from build123d import *

# Parameters (mm, degrees)
EXTRUDE_1_DEPTH     = 2
SKETCH_3_W          = 35
SKETCH_3_H          = 2
EXTRUDE_2_DEPTH     = 18
CUT_EXTRUDE_1_REACH = 87.112
SKETCH_4_R          = 2.5


with BuildPart() as part:
    # 草图1 → 旋转1 (revolve)
    with BuildSketch(Plane.XY):
        Polygon((0, 30), (0, 18.550632587), (0, 0), (18, 0), (18, 30), (15, 30), (15, 26), (3, 26), (3, 30), align=None)
    revolve(axis=Axis((18, 0, 0), (-1, 0, 0)))

    # 草图2 → 凸台-拉伸1 (add)
    with BuildSketch(Plane(origin=(18, 0, 0), x_dir=(0, 0, -1), z_dir=(1, 0, 0))):
        with BuildLine():
            Line((17.5, -40), (17.5, 0))
            ThreePointArc((17.5, 0), (0, 17.5), (-17.5, 0))
            Line((-17.5, 0), (-17.5, -40))
            Line((-17.5, -40), (17.5, -40))
        make_face()
    extrude_1 = extrude(amount=EXTRUDE_1_DEPTH)

    # 草图3 → 凸台-拉伸2 (add)
    with BuildSketch(Plane(origin=(20, 0, 0), x_dir=(0, 0, -1), z_dir=(1, 0, 0))):
        with Locations((0, -39)):
            Rectangle(SKETCH_3_W, SKETCH_3_H)
    extrude_2 = extrude(amount=EXTRUDE_2_DEPTH)

    # 镜向1: 凸台-拉伸1, 凸台-拉伸2 across plane
    add(extrude_1.mirror(Plane(origin=(9, 0, 0), x_dir=(0, 0, 1), z_dir=(1, 0, 0))))
    add(extrude_2.mirror(Plane(origin=(9, 0, 0), x_dir=(0, 0, 1), z_dir=(1, 0, 0))))

    # 草图4 → 切除-拉伸1 (cut, up to next)
    with BuildSketch(Plane.XZ.offset(40), mode=Mode.PRIVATE) as cut_extrude_1_sk1:
        with Locations((-12.5, 11)):
            Circle(SKETCH_4_R)
    cut_extrude_1_tool1 = extrude(cut_extrude_1_sk1.sketch, amount=-CUT_EXTRUDE_1_REACH, mode=Mode.PRIVATE) & part.part
    # 草图4 → 切除-拉伸1 (cut, up to next)
    with BuildSketch(Plane.XZ.offset(40), mode=Mode.PRIVATE) as cut_extrude_1_sk2:
        with Locations(Location((-12.5, -11, 0), (0, 0, 180))):
            Circle(SKETCH_4_R)
    cut_extrude_1_tool2 = extrude(cut_extrude_1_sk2.sketch, amount=-CUT_EXTRUDE_1_REACH, mode=Mode.PRIVATE) & part.part
    # 草图4 → 切除-拉伸1 (cut, up to next)
    with BuildSketch(Plane.XZ.offset(40), mode=Mode.PRIVATE) as cut_extrude_1_sk3:
        with Locations((30.5, -11)):
            Circle(SKETCH_4_R)
    cut_extrude_1_tool3 = extrude(cut_extrude_1_sk3.sketch, amount=-CUT_EXTRUDE_1_REACH, mode=Mode.PRIVATE) & part.part
    # 草图4 → 切除-拉伸1 (cut, up to next)
    with BuildSketch(Plane.XZ.offset(40), mode=Mode.PRIVATE) as cut_extrude_1_sk4:
        with Locations((30.5, 11)):
            Circle(SKETCH_4_R)
    cut_extrude_1_tool4 = extrude(cut_extrude_1_sk4.sketch, amount=-CUT_EXTRUDE_1_REACH, mode=Mode.PRIVATE) & part.part
    add(cut_extrude_1_tool1.solids().sort_by_distance((-12.5, -40, 11))[0], mode=Mode.SUBTRACT)
    add(cut_extrude_1_tool2.solids().sort_by_distance((-12.5, -40, -11))[0], mode=Mode.SUBTRACT)
    add(cut_extrude_1_tool3.solids().sort_by_distance((30.5, -40, -11))[0], mode=Mode.SUBTRACT)
    add(cut_extrude_1_tool4.solids().sort_by_distance((30.5, -40, 11))[0], mode=Mode.SUBTRACT)


solid = part.part
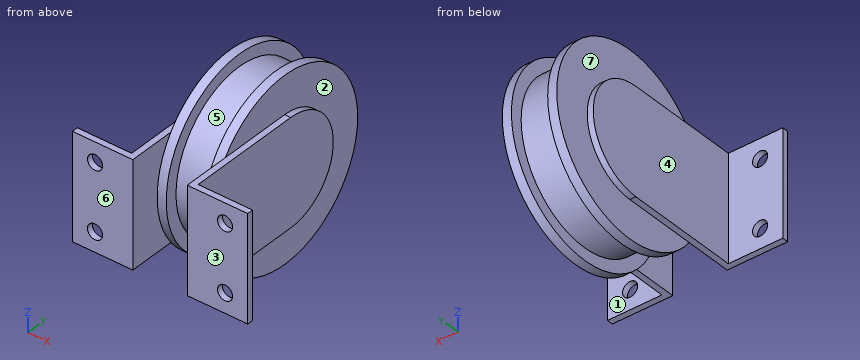
Input: part model. Units: mm. Frame: model coordinates. Face numbers are marked on the shaded views. A direction names the side the tool comes from. Give positions to 0.01 mm unless a question says otherwise; leave off trailing zeros. Write each loop counter-clockwise with the first axis right and the second up, starting at its lowest first coordinate (ties: lowest second). Pieces come first, ordered by that corner, then holes. Notation, with made-up numbers: (31, -11) -> (67, -11) arc R29 cw to (67, 18) -> close; hole circle Ø8 at (14.25, 20). An arc over 180 degrees is marked (long way). Use one line per item in the form item = value. Start each with the question number.
1) Section query C-C on y = -15.5. Return the cut outline in (x, z), then the cut area to 3 significant figures.
2) Draft query along X for the marked faces 5, 6 and 7. Return one class per face: pulls with the +X half, pulls with the -X half, needs draft (parallel to the pull), parting line crosses it, or undercut.
3) Section query D-D on z = 7. Return the cut outline in (x, y).
4) Ray query, probe 1 along Z at (x, y) = (30.5, -38.8); probe 2 along X at (y, z) = (-35, 17); probe 3 along Z at (x, y) = (30, -39). Return the intervals inside material, ascending. Write a range as from..to.
5) Pin query (flat end, axial travel): pin 1 (10 mm diameter, centred on x = 17.5, y = -2, fed in from +Z); pin 2 (17 mm diameter, centred on y = -30, z = -2.5, fed in from -X); pin 3 (5.5 mm diameter, centred on x = 26, z = 7.5, fed in from +Y); pin 4 (22 mm diameter, centred on x = -11, y = -26, fed in from +Z). Return the tip coordinate at first contact, or that it passes through.
6) Section query A-A on x = -12.5. Return the cut outline in (y, z).
7) Section query B-B on z = -11. Count the separate pieces of the cut face and the enclosed holes in it, then the cut area to 3 significant figures.
8) Set-up query: the marked faces 1, 2, 3 and 4. Return all of +Z, -Z, +X, -X, +Y, -Y with unobstructed straight access to the full face (end or side cutting, diameter ignored); none if empty.
Outcome:
q1.outline = (-2, -17.5) -> (0, -17.5) -> (0, -25.69) -> (3, -25.69) -> (3, -20.87) -> (15, -20.87) -> (15, -25.69) -> (18, -25.69) -> (18, -17.5) -> (20, -17.5) -> (20, 17.5) -> (18, 17.5) -> (18, 25.69) -> (15, 25.69) -> (15, 20.87) -> (3, 20.87) -> (3, 25.69) -> (0, 25.69) -> (0, 17.5) -> (-2, 17.5) -> close
q1.area = 949 mm^2
q2.face_5 = undercut
q2.face_6 = needs draft
q2.face_7 = pulls with the -X half
q3.outline = (-20, -40) -> (0, -40) -> (0, -29.17) -> (3, -29.17) -> (3, -25.04) -> (15, -25.04) -> (15, -29.17) -> (18, -29.17) -> (18, -40) -> (38, -40) -> (38, -38) -> (20, -38) -> (20, 16.04) -> (18, 16.04) -> (18, 29.17) -> (15, 29.17) -> (15, 25.04) -> (3, 25.04) -> (3, 29.17) -> (0, 29.17) -> (0, 16.04) -> (-2, 16.04) -> (-2, -38) -> (-20, -38) -> close
q4.probe_1 = -17.5..-13.5, -8.5..8.5, 13.5..17.5
q4.probe_2 = -2..0, 18..20
q4.probe_3 = -17.5..-13.45, -8.55..8.55, 13.45..17.5
q5.pin_1 = 30
q5.pin_2 = -20
q5.pin_3 = -38
q5.pin_4 = 17.5
q6.outline = (-40, -17.5) -> (-38, -17.5) -> (-38, -13.5) -> (-40, -13.5) -> close; (-40, -8.5) -> (-38, -8.5) -> (-38, 8.5) -> (-40, 8.5) -> close; (-40, 13.5) -> (-38, 13.5) -> (-38, 17.5) -> (-40, 17.5) -> close
q7.separate_pieces = 3
q7.enclosed_holes = 0
q7.area = 1,170 mm^2
q8.face_1 = +Z, -Z, +X, +Y
q8.face_2 = +X, +Y
q8.face_3 = +Z, -Z, +X, -X, -Y
q8.face_4 = +Z, -Z, -X, +Y
